Design review of the part built by this model. Coordinates are the model's own, in mm. A direction names the side the tool comes from. Give positions to 0.01 mm unless a question says otherwise; leave off trailing zeros. Loops run counter-clockwise (first coordinate to the right, second up) from the corner with the lowest first, then second, coordinate; pieces in that order, holes last. Notation, with made-up numbers: (77, 86.25) - (111, 86.25) arc R26 ccw to (111, 123.25) - close; hole circle Ø2 at (8, -38.5). An arc over 180 degrees is marked (long way). Write each question's results on one line, items separated by ' | '.
```python
from build123d import *

# Parameters (mm, degrees)
SKETCH_1_R             = 10
EXTRUDE_1_DEPTH        = 10
SKETCH_2_R             = 0.5
CUT_EXTRUDE_1_DEPTH    = 18.320508076
HOLE_WIZARD_M3_1_D     = 2.5
HOLE_WIZARD_M3_1_DEPTH = 8
HOLE_WIZARD_M3_2_D     = 2.5


with BuildPart() as part:
    # 草图1 → 凸台-拉伸1 (new body)
    with BuildSketch(Plane.XY):
        with Locations(Location((0, 0, 0), (0, 0, 270))):
            Circle(SKETCH_1_R)
        with BuildLine():
            Line((-1.5, 2), (1.5, 2))
            ThreePointArc((1.5, 2), (0, -2.5), (-1.5, 2))
        make_face(mode=Mode.SUBTRACT)
    extrude(amount=EXTRUDE_1_DEPTH)

    # 草图2 → 切除-拉伸1 (cut, through all)
    with BuildSketch(Plane.XY.offset(10)):
        with Locations((0, -6)):
            Circle(SKETCH_2_R)
    extrude(amount=-CUT_EXTRUDE_1_DEPTH, mode=Mode.SUBTRACT)

    # M3 螺纹孔1
    with Locations(Plane(origin=(234.411749502, 10, 915.569975215), x_dir=(-1, 0, 0), z_dir=(0, 1, 0))):
        with Locations((234.411749502, -910.569975215)):
            Hole(HOLE_WIZARD_M3_1_D / 2, depth=HOLE_WIZARD_M3_1_DEPTH)

    # M3 螺纹孔2 (through all)
    with Locations(Plane(origin=(0, 0, 0), x_dir=(-1, 0, 0), z_dir=(0, 0, -1))):
        with Locations((0, -6)):
            Hole(HOLE_WIZARD_M3_2_D / 2)


solid = part.part
```
Item 1: We need section C-C on z = 7.75. Give the boundary of the cut face in (x, y).
Output values:
outline: circle Ø20 at (0, 0); hole (-1.5, 2) arc R2.5 ccw (long way) to (1.5, 2) - close; hole circle Ø2.5 at (0, -6)
Item 2: We need section A-A on x = 0. Give the boundary of the cut face in (y, z), then the cut area to 3 significant figures.
Output values:
outline: (-10, 0) - (-7.25, 0) - (-7.25, 10) - (-10, 10) - close; (-4.75, 0) - (-2.5, 0) - (-2.5, 10) - (-4.75, 10) - close; (2, 0) - (10, 0) - (10, 3.75) - (2, 3.75) - close; (2, 6.25) - (10, 6.25) - (10, 10) - (2, 10) - close | area: 110 mm²
Item 3: Tool access review of faces 4 (the face through (0.1, 2.4, 10)), 5 (the face through (-0.27, 5.94, 3.78)), 6 (the face through (-1, 2, 4)): name each direction out of +Z, -Z, +X, -X, +Y, -Y from which nothing blocks a thin tool from reaching the whole face with its end or side.
Output values:
face 4: +Z, +X, -X, +Y, -Y | face 5: +Y | face 6: +Z, -Z
Item 4: Clearance check with flat-ended pins moving along their axes: P1, Ø6, axis at x = 1.5, z = 8.5, coming from the +Y side; P2, Ø1.5, axis at x = 6.5, z = 7, coming from the +Y side. State where each tip first meets the part, or that it passes through.
Output values:
P1: stops at y = 10 | P2: stops at y = 8.18
Item 5: Draft analysis for pull direction X (two halves, no side actions). For faces 1 (the face through (0.1, -2.5, 4.9)), 2 (the face through (0.1, 2.4, 0)), 3 (the face through (3, -9.54, 4.93)), state which applies: +X half, -X half, draft (parallel to the pull), parting line (faces both ways), or undercut.
Output values:
face 1: undercut | face 2: draft | face 3: parting line
Item 6: We need section B-B on y = -6. Give the boundary of the cut face in (x, z).
Output values:
outline: (-8, 0) - (-1.25, 0) - (-1.25, 10) - (-8, 10) - close; (1.25, 0) - (8, 0) - (8, 10) - (1.25, 10) - close
Item 7: Wall thickness on probe 1 along Y at (x, z) = (0, 3); probe 2 along Y at (x, z) = (0, 5.5); probe 3 along X at (y, z) = (0, 6.5): over which ranges is each line inside the solid? List them lowest first.
Output values:
probe 1: y = -10 to -7.25, -4.75 to -2.5, 2 to 10 | probe 2: y = -10 to -7.25, -4.75 to -2.5 | probe 3: x = -10 to -2.5, 2.5 to 10
Item 8: We need section D-D on z = 5. Give the boundary of the cut face in (x, y), then the cut area to 3 significant figures.
Output values:
outline: (-1.5, 2) - (-1.25, 2) - (-1.25, 9.92) arc R10 ccw (long way) to (1.25, 9.92) - (1.25, 2) - (1.5, 2) arc R2.5 cw (long way) to start; hole circle Ø2.5 at (0, -6) | area: 271 mm²
